from build123d import *

# Parameters (mm, degrees)
BASE_BODY_DEPTH              = 50
SIDE_WINDOW_SKETCH_W         = 30
SIDE_WINDOW_SKETCH_H         = 29
SIDE_WINDOW_CUT_DEPTH        = 107.395488626
CYLINDRICAL_BOSS_40_SKETCH_R = 20
CYLINDRICAL_BOSS_40_DEPTH    = 30
TOP_KEY_DEPTH                = 15
HOLE_16_SKETCH_R             = 8
HOLE_16_DEPTH                = 153.165355608


with BuildPart() as part:
    # Base Body Profile Sketch → Base Body (new body)
    with BuildSketch(Plane.XY):
        Polygon((0, 0), (30, 0), (30, -10), (60, -10), (60, 0), (90, 0), (90, 10), (70, 70), (20, 70), (0, 10), align=None)
    extrude(amount=-BASE_BODY_DEPTH)

    # Side Window Sketch → Side Window Cut (cut, through all)
    with BuildSketch(Plane(origin=(84, 28, 0), x_dir=(0, 0, -1), z_dir=(0.948683298050514, 0.31622776601683783, 0))):
        with Locations((25, 18.771887242)):
            Rectangle(SIDE_WINDOW_SKETCH_W, SIDE_WINDOW_SKETCH_H)
    extrude(amount=-SIDE_WINDOW_CUT_DEPTH, mode=Mode.SUBTRACT)

    # Cylindrical Boss Ø40 Sketch → Cylindrical Boss Ø40 (add)
    with BuildSketch(Plane(origin=(0, 70, 0), x_dir=(1, 0, 0), z_dir=(0, 1, 0))):
        with Locations(Location((45, 25, 0), (0, 0, 270))):
            Circle(CYLINDRICAL_BOSS_40_SKETCH_R)
    extrude(amount=CYLINDRICAL_BOSS_40_DEPTH)

    # Top Key Sketch → Top Key (add)
    with BuildSketch(Plane(origin=(0, 100, 0), x_dir=(1, 0, 0), z_dir=(0, 1, 0))):
        Polygon((25, 25), (26.66969722, 33), (63.33030278, 33), (65, 25), (63.33030278, 17), (26.66969722, 17), align=None)
    extrude(amount=TOP_KEY_DEPTH)

    # Hole Ø16 Sketch → Hole Ø16 (cut, through all)
    with BuildSketch(Plane(origin=(-1.350889359, 4.052668078, 0), x_dir=(0.9486832980505139, 0.31622776601683794, 0), z_dir=(-0.31622776601683794, 0.9486832980505139, 0))):
        with Locations(Location((76.109609582, 25, 0), (0, 0, 180))):
            Circle(HOLE_16_SKETCH_R)
    extrude(amount=-HOLE_16_DEPTH, mode=Mode.SUBTRACT)


solid = part.part
For this review, take the finished solid that the model builds, in its own axes (mm). A direction names the side the tool comes from. Coordinates: 2 decimals unless noted, no trailing zeros. Loops run counter-clockwise (first coordinate to the right, second up) from the corner with the lowest first, then second, coordinate; pieces in that order, holes last. Notation, with made-up numbers: (41, -32.75) - (65, -32.75) arc R19 ccw to (65, 1.25) - close; hole circle Ø8 at (-39, 20.25). An arc over 180 degrees is marked (long way). Use a Markdown table: item, result. Add a question column.
Item 1: Mouldability with a two-part tool opening along Z and no side actions: class faces 4 (the face through (25.847, 107.395, -20.944)), 5 (the face through (45, 107, -33)), 6 (the face through (41.9, 18.47, -24.79)) as pulls with the +Z half, pulls with the -Z half, needs draft (parallel to the pull), parting line crosses it, or undercut.
Item 2: We need section A-A (x = 14.5). Give the boundary of the cut face in (y, z).
Item 3: Tool access review of faces 1 (the face through (45, 107, -17)), 2 (the face through (25.823, 107.395, -28.944)), 3 (the face through (64.153, 107.395, -29.056)): name each direction out of +Z, -Z, +X, -X, +Y, -Y from which nothing blocks a thin tool from reaching the whole face with its end or side.
Item 4: We need section B-B (z = -14). Give the boundary of the cut face in (x, y).
Item 5: Insertion check: pin 1 Ø11 at (y, z) = (-6, -13) entering from -X; pin 2 Ø6 at (x, z) = (62, -42.5) entering from +Y; pin 3 Ø6 at (y, z) = (46.5, -43) entering from -X. Each pin has a flat end and moves straight along its axis. Give the tip position at first contact, or say it passes through.
Item 6: We need section D-D (y = 41). Give the boundary of the cut face in (x, z).
Item 7: We need section C-C (z = -21). Give the boundary of the cut face in (x, y).
Item 8: For line 1 (Z direction, x = 65, y = 51); line 2 (Y direction, x = 62, z = -4.5); line 3 (Y direction, x = 76.5, z = -13.5), list the stretches that pass through material, from the lowest coordinate up.
Results list:
| question | item | result |
|---|---|---|
| 1 | face 4 | pulls with the +Z half |
| 1 | face 5 | pulls with the -Z half |
| 1 | face 6 | undercut |
| 2 | outline | (0, -50) - (53.5, -50) - (53.5, 0) - (0, 0) - close; hole (9.34, -40) - (39.9, -40) - (39.9, -10) - (9.34, -10) - close |
| 3 | face 1 | +Z, +X, -X, +Y |
| 3 | face 2 | -Z, -X, +Y |
| 3 | face 3 | -Z, +X, +Y |
| 4 | outline | (0, 0) - (30, 0) - (30, -10) - (60, -10) - (60, 0) - (90, 0) - (90, 10) - (82.65, 32.05) - (0, 4.5) - close; (9.4, 38.21) - (73.48, 59.56) - (70, 70) - (61.7, 70) - (61.7, 100) - (28.3, 100) - (28.3, 70) - (20, 70) - close |
| 5 | pin 1 | stops at x = 30 |
| 5 | pin 2 | stops at y = 70 |
| 5 | pin 3 | stops at x = 11.17 |
| 6 | outline | (10.33, -50) - (79.67, -50) - (79.67, -40) - (17.79, -40) - (17.79, -10) - (79.67, -10) - (79.67, 0) - (10.33, 0) - close |
| 7 | outline | (0, 0) - (30, 0) - (30, -10) - (60, -10) - (60, 0) - (72.92, 0) - (64.28, 25.93) - (0, 4.5) - close; (9.4, 38.21) - (73.48, 59.56) - (70, 70) - (64.6, 70) - (64.6, 100) - (64.17, 100) - (64.17, 115) - (25.83, 115) - (25.83, 100) - (25.4, 100) - (25.4, 70) - (20, 70) - close; (77.43, 30.31) - (87.53, 0) - (90, 0) - (90, 10) - (82.65, 32.05) - close |
| 8 | line 1 | z = -50 to -40, -10 to 0 |
| 8 | line 2 | y = 0 to 70 |
| 8 | line 3 | y = 0 to 30 |
